Check sheet for the modelled part. Datum: model origin and axes. Units: mm. Give positions to 0.01 mm unless a question says otherwise; leave off trailing zeros. Order: outer loops, then holes, each group sorted by start corner. A loop starts at its lowest first (then second) coordinate and runs counter-clockwise, first axis right, second up.
from build123d import *

# Parameters (mm, degrees)
SKETCH1_R           = 25
SKETCH1_W           = 101
SKETCH1_H           = 201
BOSS_EXTRUDE1_DEPTH = 8


with BuildPart() as part:
    # Sketch1 → Boss-Extrude1 (new, symmetric)
    with BuildSketch(Plane.XY):
        with BuildLine():
            Line((80, 365), (-80, 365))
            Line((-80, 365), (-80, 125))
            Line((-80, 125), (-59.298088401, -9.150776577))
            ThreePointArc((-59.298088401, -9.150776577), (-39.057351455, -45.546935103), (0, -60))
            ThreePointArc((0, -60), (39.057351455, -45.546935103), (59.298088401, -9.150776577))
            Line((59.298088401, -9.150776577), (80, 125))
            Line((80, 125), (80, 365))
        make_face()
        Circle(SKETCH1_R, mode=Mode.SUBTRACT)
        with Locations((0, 244.5)):
            Rectangle(SKETCH1_W, SKETCH1_H, mode=Mode.SUBTRACT)
    extrude(amount=BOSS_EXTRUDE1_DEPTH, both=True)


solid = part.part
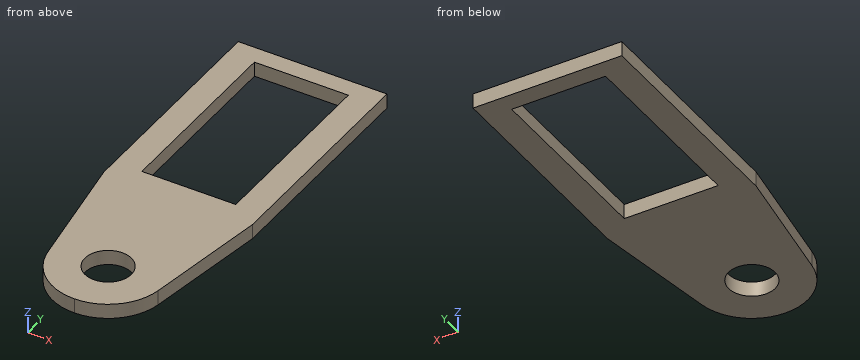
1) Section check C-C, the plane x = 19. Record the cut outline in (y, z).
Recorded:
outline: (-56.91, -8) - (-16.25, -8) - (-16.25, 8) - (-56.91, 8) - close; (16.25, -8) - (144, -8) - (144, 8) - (16.25, 8) - close; (345, -8) - (365, -8) - (365, 8) - (345, 8) - close
2) Depth check by flat-ended pin: pin 1 Ø1 at (y, z) = (14, 5) entering from -X. Enter the tip coordinate at first touch or a pass-through.
Recorded:
pin 1: stops at x = -62.95
3) Material ranges on L1, parallel to X at y = 235, z = -0.25; L2, parallel to Y at x = 16, z = -6; L3, parallel to Y at x = -21.5, z = 3.75, recorded low to high.
Recorded:
L1: x = -80 to -50.5, 50.5 to 80
L2: y = -57.83 to -19.21, 19.21 to 144, 345 to 365
L3: y = -56.02 to -12.76, 12.76 to 144, 345 to 365
4) Section check D-D, the plane x = 67. Record the cut outline in (y, z).
Recorded:
outline: (40.76, -8) - (365, -8) - (365, 8) - (40.76, 8) - close
5) Section check B-B, the plane y = 0. Record the cut outline in (x, z).
Recorded:
outline: (-60.71, -8) - (-25, -8) - (-25, 8) - (-60.71, 8) - close; (25, -8) - (60.71, -8) - (60.71, 8) - (25, 8) - close
6) Section check A-A, the plane z = 2. Record the cut outline in (x, y), then the cut area to 3 significant figures.
Recorded:
outline: (-80, 125) - (-59.3, -9.15) arc R60 ccw to (59.3, -9.15) - (80, 125) - (80, 365) - (-80, 365) - close; hole (-50.5, 144) - (50.5, 144) - (50.5, 345) - (-50.5, 345) - close; hole circle Ø50 at (0, 0)
area: 39,400 mm2
